Geometry: see drawing. Coordinates: mm, zero at the bounding-box minimum. A direction names the side the tool comes from. Give positions to 0.01 mm unless a question says otherwise; leave off trailing zeros. Write each loop counter-clockwise with the first axis right and the second up, starting at its lowest first coordinate (ties: lowest second). Pieces come first, ordered by that corner, then holes. Notation, with made-up numbers: (46.5, 25) -> (59.5, 25) arc R32 cw to (59.5, 61) -> close; hole circle Ø2 at (3, 39.5). An arc over 180 degrees is marked (long way). Answer as a JSON object with one key per item and string values. Group by question number.
Item 1: Section query A-A on x = 4. Return the cut outline in (y, z).
Item 2: Ray query, probe 1 along Z at (x, y) = (5.5, 115); probe 2 along X at (y, z) = (106, 12); probe 3 along Z at (x, y) = (18.75, 131). Return the intervals inside material, ascending. Write a range as from..to.
Item 3: Section query B-B on z = 10. Return the cut outline in (x, y), plus the area to 3 significant figures.
Item 4: Section query D-D on y = 62. Return the cut outline in (x, z).
Item 5: First-contact query: pin 1 Ø10 at (y, z) = (19.5, 15.5) entering from +X; pin 2 Ø8 at (y, z) = (98.5, 13.5) entering from -X; pin 3 Ø4 at (x, y) = (2, 112.5) entering from +Z. Flat tips, straight axial feed; report the tip coordinate or a pass-through.
Item 6: Access query for the marked faces 1, 2 and 3. Directions: +Z, -Z, +X, -X, +Y, -Y. A direction counts if a zero-diameter tool reaches every point of the face in a straight line with its end or side. Return the directions, or none.
Item 7: Section query C-C on y = 115. Return the cut outline in (x, z), plus the area to 3 significant figures.
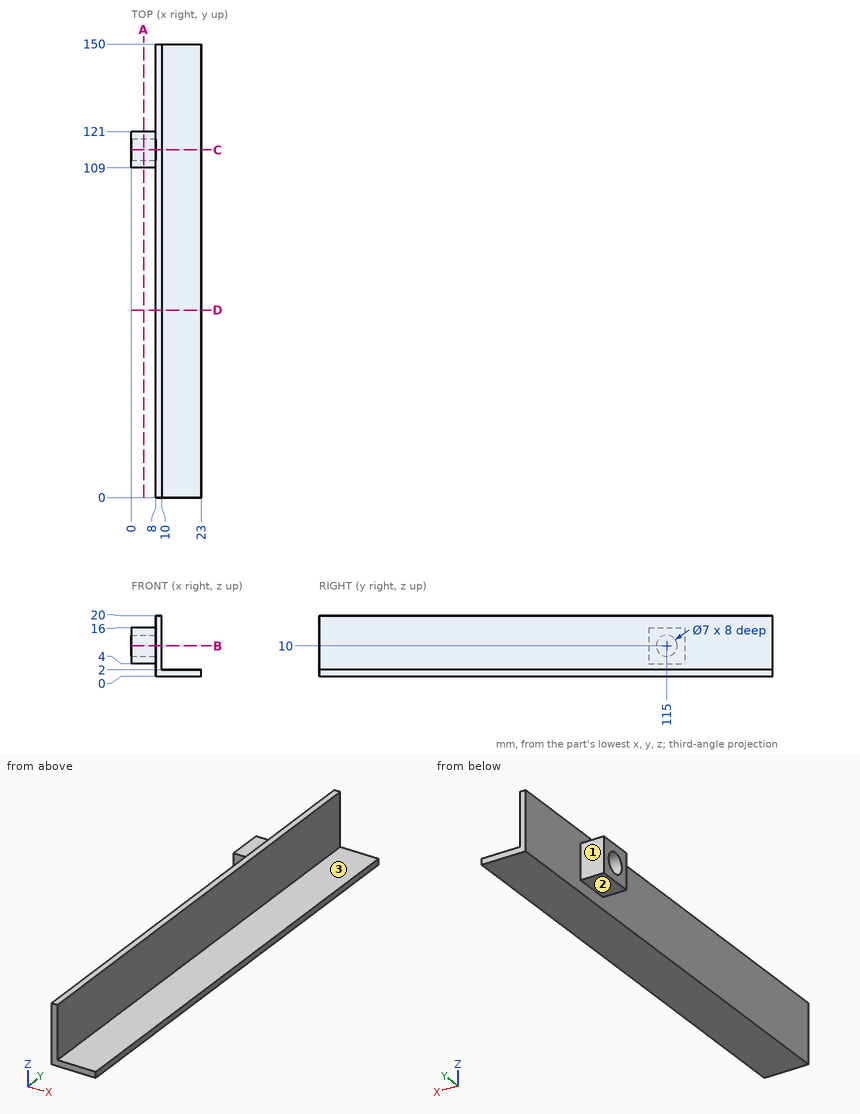
Worked answers:
{
 "1": {"outline": "(109, 4) -> (121, 4) -> (121, 16) -> (109, 16) -> close; hole circle Ø7 at (115, 10)"},
 "2": {"probe 1": "4..6.5, 13.5..16", "probe 2": "8..10", "probe 3": "0..2"},
 "3": {"outline": "(0, 109) -> (8, 109) -> (8, 0) -> (10, 0) -> (10, 150) -> (8, 150) -> (8, 121) -> (0, 121) -> (0, 118.5) -> (8, 118.5) -> (8, 111.5) -> (0, 111.5) -> close", "area": "340 mm^2"},
 "4": {"outline": "(8, 0) -> (23, 0) -> (23, 2) -> (10, 2) -> (10, 20) -> (8, 20) -> close"},
 "5": {"pin 1": "x = 10", "pin 2": "x = 8", "pin 3": "z = 16"},
 "6": {"face 1": "+Z, -Z, -X, +Y", "face 2": "-Z, -X, +Y, -Y", "face 3": "+Z, +X, +Y, -Y"},
 "7": {"outline": "(0, 4) -> (8, 4) -> (8, 0) -> (23, 0) -> (23, 2) -> (10, 2) -> (10, 20) -> (8, 20) -> (8, 16) -> (0, 16) -> (0, 13.5) -> (8, 13.5) -> (8, 6.5) -> (0, 6.5) -> close", "area": "106 mm^2"}
}
